Could you check a few things on this model? Use its own coordinates, in mm. Give positions to 0.01 mm unless a question says otherwise; leave off trailing zeros. Loops run counter-clockwise (first coordinate to the right, second up) from the corner with the lowest first, then second, coordinate; pieces in that order, holes last. Notation, with made-up numbers: (55.25, 0) - (72.25, 0) arc R11 cw to (72.25, 4) - close; hole circle Ø3 at (29.5, 36.5). An arc over 180 degrees is marked (long way). Use CSV: the item, a comma, the result in double quotes.
from build123d import *

# Parameters (mm, degrees)
SKETCH_1_W          = 222
SKETCH_1_H          = 100
EXTRUDE_1_DEPTH     = 20
SKETCH_4_R          = 3.5
CUT_EXTRUDE_1_DEPTH = 124.37341691


with BuildPart() as part:
    # 草图1 → 凸台-拉伸1 (new body)
    with BuildSketch(Plane.XY):
        Rectangle(SKETCH_1_W, SKETCH_1_H)
    extrude(amount=EXTRUDE_1_DEPTH)

    # 草图4 → 切除-拉伸1 (cut, through all)
    with BuildSketch(Plane.XY.offset(20)):
        with Locations((-101, 19)):
            Circle(SKETCH_4_R)
        with Locations((-101, -40)):
            Circle(SKETCH_4_R)
        with Locations((101, 19)):
            Circle(SKETCH_4_R)
        with Locations((101, -40)):
            Circle(SKETCH_4_R)
    extrude(amount=-CUT_EXTRUDE_1_DEPTH, mode=Mode.SUBTRACT)


solid = part.part
1) I need wall thicknesses on line 1 along Y through (x, z) = (101, 13.25); line 2 along X through (y, z) = (-38, 17.75); line 3 along X through (y, z) = (-41.5, 16.25). Which ranges of each line are inside material? Lowest first, please.
Answer below:
line 1,"y = -50 to -43.5, -36.5 to 15.5, 22.5 to 50"
line 2,"x = -111 to -103.87, -98.13 to 98.13, 103.87 to 111"
line 3,"x = -111 to -104.16, -97.84 to 97.84, 104.16 to 111"
2) Suppose I cut it at A-A (y = -40). Please give me the cut outline in (x, z).
Answer below:
outline,"(-111, 0) - (-104.5, 0) - (-104.5, 20) - (-111, 20) - close; (-97.5, 0) - (97.5, 0) - (97.5, 20) - (-97.5, 20) - close; (104.5, 0) - (111, 0) - (111, 20) - (104.5, 20) - close"
3) We'd pull the mould along X, two halves only. Please class faces 1 (the cylindrical face through (104.34, -38.95, 10.14)), 2 (the flat face through (-111, -1, 10)), 3 (the flat face through (-2, 1, 0)): +X half, -X half, draft (parallel to the pull), parting line (faces both ways), or undercut.
Answer below:
face 1,"undercut"
face 2,"-X half"
face 3,"draft"
4) Suppose I cut it at B-B (x = 101). Please give me the cut outline in (y, z), plus the area to 3 significant figures.
Answer below:
outline,"(-50, 0) - (-43.5, 0) - (-43.5, 20) - (-50, 20) - close; (-36.5, 0) - (15.5, 0) - (15.5, 20) - (-36.5, 20) - close; (22.5, 0) - (50, 0) - (50, 20) - (22.5, 20) - close"
area,"1,720 mm2"
5) I'm going to push flat-ended pins straight in: P1, Ø1.5, axis at x = 0.5, y = -26.5, coming from the -Z side; P2, Ø5.5, axis at x = 101, y = -40, coming from the +Z side. Where does each tip first touch, or does it pass through?
Answer below:
P1,"stops at z = 0"
P2,"passes through"
